Could you check a few things on this model? Use its own coordinates, in mm. A direction names the side the tool comes from. Coordinates: 2 decimals unless noted, no trailing zeros. Order: outer loops, then holes, each group sorted by start corner. A loop starts at its lowest first (then second) coordinate and runs counter-clockwise, first axis right, second up. Notation, with made-up numbers: (-32, 65.25) -> (15, 65.25) arc R10 ccw to (15, 77.25) -> close; hole circle Ø2 at (13.25, -10). An arc over 180 degrees is marked (long way). Return JSON: item names as keys, results as strings. Group by question number.
from build123d import *

# Parameters (mm, degrees)
GB_T_707_1988_HOT_ROLLED_CHANNEL_05_1_DEPTH = 760


with BuildPart() as part:
    # Sketch1 → GB/T 707-1988 hot-rolled channel 05(1) (new body)
    with BuildSketch(Plane.YZ.offset(-380)):
        with BuildLine():
            Line((37, 50), (0, 50))
            Line((0, 50), (0, 0))
            Line((0, 0), (37, 0))
            Line((37, 0), (37, 2.140642022))
            ThreePointArc((37, 2.140642022), (36.101006889, 4.482599144), (33.865849621, 5.621468656))
            Line((33.865849621, 5.621468656), (10.768300757, 8.049118866))
            ThreePointArc((10.768300757, 8.049118866), (6.297986222, 10.326857889), (4.5, 15.010772133))
            Line((4.5, 15.010772133), (4.5, 34.989227867))
            ThreePointArc((4.5, 34.989227867), (6.297986222, 39.673142111), (10.768300757, 41.950881134))
            Line((10.768300757, 41.950881134), (33.865849621, 44.378531344))
            ThreePointArc((33.865849621, 44.378531344), (36.101006889, 45.517400856), (37, 47.859357978))
            Line((37, 47.859357978), (37, 50))
        make_face()
    extrude(amount=GB_T_707_1988_HOT_ROLLED_CHANNEL_05_1_DEPTH)


solid = part.part
Q1. I'm going to push flat-ended pins straight in: pin 1 Ø16 at (x, z) = (-100, 29.5) entering from +Y; pin 2 Ø12 at (x, z) = (81.5, 11.5) entering from -Y; pin 3 Ø8 at (y, z) = (10.5, 21) entering from -X. Where does each tip first touch, or does it pass through?
Q2. We'd pull the mould along X, two halves only. Please class faces 3 (the flat face through (380, 3, 23)), 4 (the flat face through (-380, 3, 23)), 5 (the flat face through (-5, 0, 25)): pulls with the +X half, pulls with the -X half, needs draft (parallel to the pull), parting line crosses it, or undercut.
Q3. I want a section at A-A on y = 25. Please give me the cut outline in (x, z).
Q4. I want a section at B-B on x = -238.5. Please give me the cut outline in (y, z).
Q5. I want a section at C-C on z = 27. Please give me the cut outline in (x, y).
Q6. On a 3-axis mill with a long thin cutter (end or side, diameter ignored), from which of +Z, -Z, +X, -X, +Y, -Y can I reach the whole of each face in a straight line? I mean faces 1 (the flat face through (-5.32, 22.16, 43.15)), 2 (the flat face through (-5, 19, 50)). Say none if no direction works.
Q7. I need wall thicknesses on line 1 along Z through (x, y) = (-283, 20.5); line 2 along Z through (x, y) = (347, 11); line 3 along Y through (x, z) = (43, 20.5). Which ranges of each line are inside material? Lowest first, please. Write a range as from..to.
Response values:
{
 "1": {"pin 1": "stops at y = 4.97", "pin 2": "stops at y = 0", "pin 3": "passes through"},
 "2": {"face 3": "pulls with the +X half", "face 4": "pulls with the -X half", "face 5": "needs draft"},
 "3": {"outline": "(-380, 0) -> (380, 0) -> (380, 6.55) -> (-380, 6.55) -> close; (-380, 43.45) -> (380, 43.45) -> (380, 50) -> (-380, 50) -> close"},
 "4": {"outline": "(0, 0) -> (37, 0) -> (37, 2.14) arc R3.5 ccw to (33.87, 5.62) -> (10.77, 8.05) arc R7 cw to (4.5, 15.01) -> (4.5, 34.99) arc R7 cw to (10.77, 41.95) -> (33.87, 44.38) arc R3.5 ccw to (37, 47.86) -> (37, 50) -> (0, 50) -> close"},
 "5": {"outline": "(-380, 0) -> (380, 0) -> (380, 4.5) -> (-380, 4.5) -> close"},
 "6": {"face 1": "+X, -X, +Y", "face 2": "+Z, +X, -X, +Y, -Y"},
 "7": {"line 1": "z = 0..7.03, 42.97..50", "line 2": "z = 0..8.02, 41.98..50", "line 3": "y = 0..4.5"}
}
